Model file for the job. Use its own axes, mm. A direction names the side the tool comes from. Round coordinates to 2 decimals unless told otherwise and drop trailing zeros. Loops run counter-clockwise (first coordinate to the right, second up) from the corner with the lowest first, then second, coordinate; pieces in that order, holes last. Notation, with made-up numbers: M -28.5,-9.75 L 10.5,-9.75 A7 ccw 10.5,-4.75 Z; hole C 62,40.5 d10. An arc over 180 degrees is marked long. Use a Markdown table: item, result. Add a question column.
Q1. Tool access for faces 1 (the face through (-2, 0, 0)), 2 (the face through (-2, -1.5, 13)), 3 (the face through (-2, 1.5, 13)): list every direction of +Z, -Z, +X, -X, +Y, -Y with a clear straight run to the whole face (end or side of a thin tool).
Q2. Cut at C-C (z = 14). Give the cut face in (x, y).
Q3. Cut at A-A (y = 0.4). Give the cut face in (x, z), plus the area to 3 significant figures.
Q4. Probe line 1 (Y direction, x = 67.5, z = 18); line 2 (Z direction, x = 111.5, y = 1.6); line 3 (X direction, y = 0, z = 11.25). List the from-to ranges inside material, lowest first. Write a range as from..to.
Q5. Pin check, flat tips, straight feed: pin 1 (3 mm diameter, centred on y = 1, z = 12.5, fed in from +X); pin 2 (4.5 mm diameter, centred on x = -54, z = 13, fed in from -Y); pin 3 (1 mm diameter, centred on x = 21.5, z = 14, fed in from +Y). Stop position of each tip, or through.
Q6. Cut at B-B (x = 98). Give the cut face in (y, z), plus the area to 3 significant figures.
from build123d import *

# Parameters (mm, degrees)
SKETCH1_W           = 313
SKETCH1_H           = 5
BOSS_EXTRUDE1_DEPTH = 5.5
CUT_EXTRUDE1_DEPTH  = 314.058301279
SKETCH2_W           = 283
SKETCH2_H           = 3
BOSS_EXTRUDE2_DEPTH = 15


with BuildPart() as part:
    # Sketch1 → Boss-Extrude1 (new body)
    with BuildSketch(Plane.XY):
        Rectangle(SKETCH1_W, SKETCH1_H)
    extrude(amount=BOSS_EXTRUDE1_DEPTH)

    # Sketch3 → Cut-Extrude1 (cut, through all)
    with BuildSketch(Plane(origin=(156.5, 0, 0), x_dir=(0, 0, -1), z_dir=(1, 0, 0))):
        Polygon((-3, 2.5), (-5.5, 1.75), (-5.5, 2.5), align=None)
        Polygon((-3, -2.5), (-5.5, -1.75), (-5.5, -2.5), align=None)
    extrude(amount=-CUT_EXTRUDE1_DEPTH, mode=Mode.SUBTRACT)

    # Sketch2 → Boss-Extrude2 (add)
    with BuildSketch(Plane.XY.offset(5.5)):
        Rectangle(SKETCH2_W, SKETCH2_H)
    extrude(amount=BOSS_EXTRUDE2_DEPTH)


solid = part.part
Checked values:
| question | item | result |
|---|---|---|
| 1 | face 1 | -Z, +X, -X, +Y, -Y |
| 1 | face 2 | +Z, +X, -X, -Y |
| 1 | face 3 | +Z, +X, -X, +Y |
| 2 | outline | M -141.5,-1.5 L 141.5,-1.5 L 141.5,1.5 L -141.5,1.5 Z |
| 3 | outline | M -156.5,0 L 156.5,0 L 156.5,5.5 L 141.5,5.5 L 141.5,20.5 L -141.5,20.5 L -141.5,5.5 L -156.5,5.5 Z |
| 3 | area | 5,970 mm^2 |
| 4 | line 1 | y = -1.5..1.5 |
| 4 | line 2 | z = 0..5.5 |
| 4 | line 3 | x = -141.5..141.5 |
| 5 | pin 1 | stops at x = 141.5 |
| 5 | pin 2 | stops at y = -1.5 |
| 5 | pin 3 | stops at y = 1.5 |
| 6 | outline | M -2.5,0 L 2.5,0 L 2.5,3 L 1.75,5.5 L 1.5,5.5 L 1.5,20.5 L -1.5,20.5 L -1.5,5.5 L -1.75,5.5 L -2.5,3 Z |
| 6 | area | 70.6 mm^2 |
